Geometry: final body of the model. Coordinates: model frame, mm. A direction names the side the tool comes from. Round coordinates to 2 decimals unless told otherwise and drop trailing zeros. Order: outer loops, then holes, each group sorted by start corner. A loop starts at its lowest first (then second) coordinate and runs counter-clockwise, first axis right, second up. Notation, with made-up numbers: (53, -34) - (60, -34) arc R10 ccw to (60, -16) - close; hole circle Ø7 at (-1, 11.25). An arc over 180 degrees is marked (long way). Put each result on its own line as item: value. Start each with the question number.
(1) Section A-A (y = 0). Output: boundary loops of the cut face in (x, z).
(2) Section D-D (x = -4.25). Output: boundary loops of the cut face in (y, z).
(3) Section C-C (z = 5). Output: boundary loops of the cut face in (x, y), and give its area (3 significant figures).
(4) Access query for faces 1 (the face through (4.8, -8, -5)), 2 (the face through (0, 5.4, 8)), 3 (the face through (-4.8, -8, -5)). Directions: +Z, -Z, +X, -X, +Y, -Y. A direction counts if a zero-diameter tool reaches every point of the face in a straight line with its end or side. Return the directions, or none.
(5) Pin query (flat end, axial travel): P1, Ø2.5, axis at x = 0, z = 8, coming from the -Y side; P2, Ø1.4, axis at y = -7.5, z = -5.5, coming from the +X side; P3, Ø8, axis at x = -10, z = 0.5, coming from the +Y side. Return the tip coordinate at first contact, or that it passes through.
(6) Pull-direction query (Y, two-part tool) for faces 4 (the face through (0, 4, 9.48)), 5 (the face through (9, 2.1, -1)), 6 (the face through (-9.355, 0.36, -0.887)); classes: released by +Y, released by -Y, zero draft, split by the parting line, or undercut.
(7) Material intervals for L1, parallel to Y at x = 10.5, z = -1.3; L2, parallel to Z at x = -7.75, y = 2.5; L3, parallel to X at y = 3.75, z = 3.25, sorted ascending. Write a range as [from, to].
(8) Section B-B (x = 9.75). Output: boundary loops of the cut face in (y, z).
from build123d import *

# Parameters (mm, degrees)
SKETCH_1_3_R        = 2.5
BOSS_EXTRUDE1_DEPTH = 19.2
SKETCH_1_3_2_R      = 2
BOSS_EXTRUDE2_DEPTH = 3
SKETCH2_R           = 3.5
BOSS_EXTRUDE3_DEPTH = 35
CUT_EXTRUDE1_START  = -2.5
CUT_EXTRUDE1_DEPTH  = 2.5
SKETCH6_W           = 6
SKETCH6_H           = 1
CUT_EXTRUDE2_DEPTH  = 5
SCALE1_SCALE        = 0.6


with BuildPart() as part:
    # Sketch 1_3 → Boss-Extrude1 (new body)
    # profile 1 of 3: a face of its own
    with BuildSketch(Plane.XY):
        with BuildLine():
            ThreePointArc((14, 0), (0, 14), (-14, 0))
            ThreePointArc((-14, 0), (0, -14), (14, 0))
        make_face()
        with Locations((0, 6.5)):
            Circle(SKETCH_1_3_R, mode=Mode.SUBTRACT)
    # profile 2 of 3: a face of its own
    with BuildSketch(Plane.XY):
        with BuildLine():
            Line((8, -16), (8, -11.489125293))
            ThreePointArc((8, -11.489125293), (4.192388692, -13.357540082), (0, -14))
            Line((0, -14), (0, -18))
            Line((0, -18), (6, -18))
            ThreePointArc((6, -18), (7.414213562, -17.414213562), (8, -16))
        make_face()
    # profile 3 of 3: a face of its own
    with BuildSketch(Plane.XY):
        with BuildLine():
            Line((0, -18), (0, -14))
            ThreePointArc((0, -14), (-4.192388692, -13.357540082), (-8, -11.489125293))
            Line((-8, -11.489125293), (-8, -16))
            ThreePointArc((-8, -16), (-7.414213562, -17.414213562), (-6, -18))
            Line((-6, -18), (0, -18))
        make_face()
    extrude(amount=-BOSS_EXTRUDE1_DEPTH)

    # Sketch 1_3 2 → Boss-Extrude2 (add)
    # profile 1 of 2: a face of its own
    with BuildSketch(Plane.XY):
        with BuildLine():
            ThreePointArc((-14, 0), (-13.888415748, 1.764060095), (-13.555441712, 3.5))
            Line((-13.555441712, 3.5), (-17.5, 3.5))
            ThreePointArc((-17.5, 3.5), (-21, 0), (-17.5, -3.5))
            Line((-17.5, -3.5), (-13.555441712, -3.5))
            ThreePointArc((-13.555441712, -3.5), (-13.888415748, -1.764060095), (-14, 0))
        make_face()
        with Locations((-17.5, 0)):
            Circle(SKETCH_1_3_2_R, mode=Mode.SUBTRACT)
    # profile 2 of 2: a face of its own
    with BuildSketch(Plane.XY):
        with BuildLine():
            Line((13.555441712, -3.5), (17.5, -3.5))
            ThreePointArc((17.5, -3.5), (21, 0), (17.5, 3.5))
            Line((17.5, 3.5), (13.555441712, 3.5))
            ThreePointArc((13.555441712, 3.5), (13.888415748, 1.764060095), (14, 0))
            ThreePointArc((14, 0), (13.888415748, -1.764060095), (13.555441712, -3.5))
        make_face()
        with Locations((17.5, 0)):
            Circle(SKETCH_1_3_2_R, mode=Mode.SUBTRACT)
    extrude(amount=-BOSS_EXTRUDE2_DEPTH)

    # Sketch2 → Boss-Extrude3 (add)
    with BuildSketch(Plane(origin=(0, 0, -19.2), x_dir=(-1, 0, 0), z_dir=(0, 0, -1))):
        with Locations((0, 6.5)):
            Circle(SKETCH2_R)
    extrude(amount=-BOSS_EXTRUDE3_DEPTH)

    # Sketch5 → Cut-Extrude1 (cut)
    with BuildSketch(Plane(origin=(0, 0, -19.2), x_dir=(-1, 0, 0), z_dir=(0, 0, -1)).offset(CUT_EXTRUDE1_START)):
        with BuildLine():
            Line((-8, -11.489125293), (-8, -16))
            ThreePointArc((-8, -16), (-7.414213562, -17.414213562), (-6, -18))
            Line((-6, -18), (6, -18))
            ThreePointArc((6, -18), (7.414213562, -17.414213562), (8, -16))
            Line((8, -16), (8, -11.489125293))
            ThreePointArc((8, -11.489125293), (0, -14), (-8, -11.489125293))
        make_face()
    extrude(amount=CUT_EXTRUDE1_DEPTH, mode=Mode.SUBTRACT)

    # Sketch6 → Cut-Extrude2 (cut, symmetric)
    with BuildSketch(Plane(origin=(0, 0, 0), x_dir=(0, 0, -1), z_dir=(1, 0, 0))):
        with Locations((-12.8, 9.5)):
            Rectangle(SKETCH6_W, SKETCH6_H)
        with Locations((-12.8, 3.5)):
            Rectangle(SKETCH6_W, SKETCH6_H)
    extrude(amount=CUT_EXTRUDE2_DEPTH, both=True, mode=Mode.SUBTRACT)


with BuildPart() as part_1:
    # Scale1: scaled about (0, 0, 0)
    add(part.part.scale(SCALE1_SCALE))


solid = part_1.part
Checks:
1. outline: (-12.6, -1.8) - (-11.7, -1.8) - (-11.7, 0) - (-12.6, 0) - close; (-9.3, -1.8) - (-8.4, -1.8) - (-8.4, -11.52) - (8.4, -11.52) - (8.4, -1.8) - (9.3, -1.8) - (9.3, 0) - (-9.3, 0) - close; (11.7, -1.8) - (12.6, -1.8) - (12.6, 0) - (11.7, 0) - close
2. outline: (-10.61, -10.02) - (-7.25, -10.02) - (-7.25, -11.52) - (7.25, -11.52) - (7.25, 0) - (-10.61, 0) - close
3. outline: circle Ø4.2 at (0, 3.9)
3. area: 13.9 mm²
4. face 1: +Z, -Z, +X, -Y
4. face 2: +Z, +X, -X, +Y
4. face 3: +Z, -Z, -X, -Y
5. P1: stops at y = 2.4
5. P2: stops at x = 4.93
5. P3: stops at y = 5.85
6. face 4: zero draft
6. face 5: released by +Y
6. face 6: undercut
7. L1: y = [-2.1, -1.2], [1.2, 2.1]
7. L2: z = [-11.52, 0]
7. L3: x = [-2.09, 2.09]
8. outline: (-2.1, -1.8) - (-0.94, -1.8) - (-0.94, 0) - (-2.1, 0) - close; (0.94, -1.8) - (2.1, -1.8) - (2.1, 0) - (0.94, 0) - close
